Part model, mm, in its own coordinate system. Face numbers are marked on the shaded views. A direction names the side the tool comes from. Coordinates: 2 decimals unless noted, no trailing zeros. Loops run counter-clockwise (first coordinate to the right, second up) from the corner with the lowest first, then second, coordinate; pieces in that order, holes last. Notation, with made-up numbers: (52.25, -18.5) -> (58.25, -18.5) arc R9 cw to (58.25, -2.5) -> close; hole circle Ø5 at (34.5, 42). An arc over 180 degrees is marked (long way). Use one line per item in the form item = value. Start each with the question number.
(1) Mould opens along Z. For the marked faces 1, 2, 3 and 4 say: +Z half, -Z half, draft (parallel to the pull), parting line (faces both ways), or undercut.
(2) 3-axis set-ups, long thin cutter, end or side, ignore diameter. For the marked faces 5, 6, 7, 8 and 9: which of +Z, -Z, +X, -X, +Y, -Y reach the whole face in a straight line?
(3) Drill centre lines: L1, parallel to Z at x = 67, y = 4; L2, parallel to X at y = 24, z = -20.5; L3, parallel to Z at x = 74, y = 32. Where is each one in solid material? Low to high. Write a range as [from, to].
(4) Band-saw the part on B-B on y = 12. Give the cut face in (x, z).
(5) Band-saw the part on C-C on x = 67.5. Give the cut face in (y, z), then the cut area to 3 significant figures.
(6) Band-saw the part on A-A on z = -25. Give the cut face in (x, y), then the cut area to 3 significant figures.
(7) Band-saw the part on D-D on z = -11. Give the cut face in (x, y).
(8) Pin check, flat tips, straight feed: P1, Ø8, axis at x = 17, y = -4.5, coming from the -Z side; P2, Ø8, axis at x = 48, z = -26.5, coming from the +Y side; P3, Ø2, axis at y = 24, z = -10, coming from the -X side; P4, Ø13.5, axis at x = 14.5, z = -37, coming from the +Y side. Stop position of each tip, or through.
```python
from build123d import *

# Parameters (mm, degrees)
BASE_PLATE_SKETCH_W      = 90
BASE_PLATE_SKETCH_H      = 15
BASE_PLATE_DEPTH         = 50
SIDE_WALL_SKETCH_W       = 45
SIDE_WALL_SKETCH_H       = 15
SIDE_WALL_DEPTH          = 50
RAISED_BLOCK_SKETCH_W    = 55
RAISED_BLOCK_SKETCH_H    = 20
RAISED_BLOCK_DEPTH       = 50
STEP_NOTCH_CUT_DEPTH     = 50
FIRST_ROUNDED_LUG_DEPTH  = 10
SECOND_START             = -10
SECOND_ROUNDED_LUG_DEPTH = 10
SLOT_CUT_DEPTH           = 15
CHANNEL_SKETCH_W         = 30
CHANNEL_SKETCH_H         = 20
CHANNEL_CUT_DEPTH        = 60
RAIL_BOSS_SKETCH_W       = 30
RAIL_BOSS_SKETCH_H       = 20
RAIL_BOSS_DEPTH          = 10
CURVED_RECESS_SKETCH_W   = 10
CURVED_RECESS_SKETCH_H   = 30
CURVED_RECESS_CUT_DEPTH  = 5
BRIDGE_BLOCK_SKETCH_W    = 10
BRIDGE_BLOCK_SKETCH_H    = 30
BRIDGE_BLOCK_DEPTH       = 20
BRIDGE_RELIEF_SKETCH_W   = 10
BRIDGE_RELIEF_SKETCH_H   = 30
BRIDGE_RELIEF_CUT_DEPTH  = 5
BORE_24_SKETCH_R         = 12
BORE_24_DEPTH            = 70


with BuildPart() as part:
    # Base Plate Sketch → Base Plate (new body)
    with BuildSketch(Plane.XY):
        with Locations((45, 7.5)):
            Rectangle(BASE_PLATE_SKETCH_W, BASE_PLATE_SKETCH_H)
    extrude(amount=-BASE_PLATE_DEPTH)

    # Side Wall Sketch → Side Wall (add)
    with BuildSketch(Plane.XY):
        with Locations((67.5, -7.5)):
            Rectangle(SIDE_WALL_SKETCH_W, SIDE_WALL_SKETCH_H)
    extrude(amount=-SIDE_WALL_DEPTH)

    # Raised Block Sketch → Raised Block (add)
    with BuildSketch(Plane.XY):
        with Locations((62.5, 25)):
            Rectangle(RAISED_BLOCK_SKETCH_W, RAISED_BLOCK_SKETCH_H)
    extrude(amount=-RAISED_BLOCK_DEPTH)

    # Step Notch Sketch → Step Notch Cut (cut)
    with BuildSketch(Plane(origin=(0, 15, 0), x_dir=(1, 0, 0), z_dir=(0, 1, 0))):
        with BuildLine():
            Line((10, 50), (0, 50))
            Line((0, 50), (0, 40))
            ThreePointArc((0, 40), (2.928932188, 47.071067812), (10, 50))
        make_face()
        with BuildLine():
            ThreePointArc((10, 0), (2.928932188, 2.928932188), (0, 10))
            Line((0, 10), (0, 0))
            Line((0, 0), (10, 0))
        make_face()
    extrude(amount=-STEP_NOTCH_CUT_DEPTH, mode=Mode.SUBTRACT)

    # First Rounded Lug Sketch → First Rounded Lug (add)
    with BuildSketch(Plane.XY):
        with BuildLine():
            Line((35, 35), (35, 15))
            Line((35, 15), (15, 15))
            ThreePointArc((15, 15), (29.142135624, 20.857864376), (35, 35))
        make_face()
    extrude(amount=-FIRST_ROUNDED_LUG_DEPTH)

    # Second Rounded Lug Sketch → Second Rounded Lug (add)
    with BuildSketch(Plane(origin=(0, 0, -50), x_dir=(-1, 0, 0), z_dir=(0, 0, -1)).offset(SECOND_START)):
        with BuildLine():
            Line((-35, 35), (-35, 15))
            Line((-35, 15), (-15, 15))
            ThreePointArc((-15, 15), (-29.142135624, 20.857864376), (-35, 35))
        make_face()
    extrude(amount=SECOND_ROUNDED_LUG_DEPTH)

    # Slot Sketch → Slot Cut (cut)
    with BuildSketch(Plane(origin=(0, 15, 0), x_dir=(1, 0, 0), z_dir=(0, 1, 0))):
        with BuildLine():
            Line((0, 25), (0, 31))
            Line((0, 31), (11.291796068, 31))
            ThreePointArc((11.291796068, 31), (27, 25), (11.291796068, 19))
            Line((11.291796068, 19), (0, 19))
            Line((0, 19), (0, 25))
        make_face()
    extrude(amount=-SLOT_CUT_DEPTH, mode=Mode.SUBTRACT)

    # Channel Sketch → Channel Cut (cut)
    with BuildSketch(Plane.ZY.offset(-35)):
        with Locations((-25, 25)):
            Rectangle(CHANNEL_SKETCH_W, CHANNEL_SKETCH_H)
    extrude(amount=-CHANNEL_CUT_DEPTH, mode=Mode.SUBTRACT)

    # Rail Boss Sketch → Rail Boss (add)
    with BuildSketch(Plane(origin=(90, 0, 0), x_dir=(0, 0, -1), z_dir=(1, 0, 0))):
        with Locations((25, 25)):
            Rectangle(RAIL_BOSS_SKETCH_W, RAIL_BOSS_SKETCH_H)
    extrude(amount=-RAIL_BOSS_DEPTH)

    # Curved Recess Sketch → Curved Recess Cut (cut)
    with BuildSketch(Plane(origin=(0, 35, 0), x_dir=(1, 0, 0), z_dir=(0, 1, 0))):
        with Locations((85, 25)):
            Rectangle(CURVED_RECESS_SKETCH_W, CURVED_RECESS_SKETCH_H)
    extrude(amount=-CURVED_RECESS_CUT_DEPTH, mode=Mode.SUBTRACT)

    # Bridge Block Sketch → Bridge Block (add)
    with BuildSketch(Plane(origin=(0, 35, 0), x_dir=(1, 0, 0), z_dir=(0, 1, 0))):
        with Locations((50, 25)):
            Rectangle(BRIDGE_BLOCK_SKETCH_W, BRIDGE_BLOCK_SKETCH_H)
    extrude(amount=-BRIDGE_BLOCK_DEPTH)

    # Bridge Relief Sketch → Bridge Relief Cut (cut)
    with BuildSketch(Plane(origin=(0, 35, 0), x_dir=(1, 0, 0), z_dir=(0, 1, 0))):
        with Locations((50, 25)):
            Rectangle(BRIDGE_RELIEF_SKETCH_W, BRIDGE_RELIEF_SKETCH_H)
    extrude(amount=-BRIDGE_RELIEF_CUT_DEPTH, mode=Mode.SUBTRACT)

    # Bore Ø24 Sketch → Bore Ø24 (cut)
    with BuildSketch(Plane(origin=(0, 15, 0), x_dir=(1, 0, 0), z_dir=(0, 1, 0))):
        with Locations(Location((67.5, 25, 0), (0, 0, 270))):
            Circle(BORE_24_SKETCH_R)
    extrude(amount=-BORE_24_DEPTH, mode=Mode.SUBTRACT)


solid = part.part
```
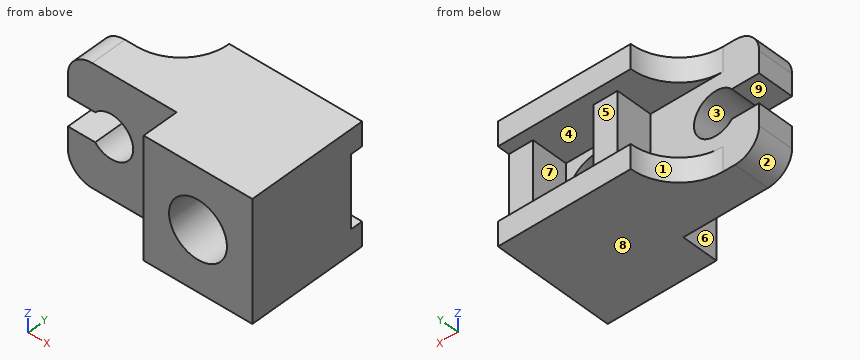
A:
q1.face_1 = draft
q1.face_2 = -Z half
q1.face_3 = undercut
q1.face_4 = undercut
q2.face_5 = +X, -X, +Y
q2.face_6 = +Z, -Z, -X, -Y
q2.face_7 = +Y
q2.face_8 = -Z, +X, -X, +Y, -Y
q2.face_9 = -X, +Y, -Y
q3.L1 = [-50, -36.99], [-13.01, 0]
q3.L2 = [45, 55], [80, 90]
q3.L3 = [-50, -40], [-10, 0]
q4.outline = (0, -40) arc R10 ccw to (10, -50) -> (90, -50) -> (90, 0) -> (10, 0) arc R10 ccw to (0, -10) -> (0, -19) -> (11.29, -19) arc R9 cw (long way) to (11.29, -31) -> (0, -31) -> close; hole circle Ø24 at (67.5, -25)
q5.outline = (-15, -50) -> (35, -50) -> (35, -40) -> (15, -40) -> (15, -37) -> (-15, -37) -> close; (-15, -13) -> (15, -13) -> (15, -10) -> (35, -10) -> (35, 0) -> (-15, 0) -> close
q5.area = 1,180 mm²
q6.outline = (27, 0) -> (45, 0) -> (45, -15) -> (55.5, -15) -> (55.5, 15) -> (55, 15) -> (55, 30) -> (45, 30) -> (45, 15) -> (27, 15) -> close; (79.5, -15) -> (90, -15) -> (90, 30) -> (80, 30) -> (80, 15) -> (79.5, 15) -> close
q6.area = 1,200 mm²
q7.outline = (0, 0) -> (45, 0) -> (45, -15) -> (90, -15) -> (90, 30) -> (80, 30) -> (80, 15) -> (55, 15) -> (55, 30) -> (45, 30) -> (45, 15) -> (0, 15) -> close
q8.P1 = through
q8.P2 = 30
q8.P3 = 31
q8.P4 = 15.78
